Input: part model. Units: mm. Frame: model coordinates. Face numbers are marked on the shaded views. A direction names the side the tool comes from. Round coordinates to 2 decimals unless told otherwise and drop trailing zeros. Order: outer loops, then holes, each group sorted by start corner. A loop starts at its lowest first (then second) coordinate and runs counter-clockwise, first axis right, second up. Notation, with made-up numbers: (-28, 85.25) -> (16, 85.25) arc R22 ccw to (16, 115.25) -> close; hole circle Ø8 at (73, -8.5). An arc over 180 degrees is marked (long way). Use a Markdown table: item, result.
from build123d import *

# Parameters (mm, degrees)
BASE_PLATE_DEPTH           = 580
MOUNTING_HOLES_SKETCH_R    = 5.7
MOUNTING_HOLES_8X_11_DEPTH = 580
HOLE_CHAMFERS_6MM_SIZE     = 9.8


with BuildPart() as part:
    # Plate Profile Sketch → Base Plate (new body)
    with BuildSketch(Plane(origin=(0, 0, 0), x_dir=(0, 0, -1), z_dir=(1, 0, 0))):
        Polygon((-68.5, 0), (68.5, 0), (68.5, 10), (124, 10), (124, 40), (-124, 40), (-124, 10), (-68.5, 10), align=None)
    extrude(amount=BASE_PLATE_DEPTH)

    # Mounting Holes Sketch → Mounting Holes 8xØ11 (cut)
    with BuildSketch(Plane(origin=(0, 40, 0), x_dir=(1, 0, 0), z_dir=(0, 1, 0))):
        with Locations(Location((25, -91.5, 0), (0, 0, 270))):
            Circle(MOUNTING_HOLES_SKETCH_R)
        with Locations(Location((157.5, -91.5, 0), (0, 0, 270))):
            Circle(MOUNTING_HOLES_SKETCH_R)
        with Locations(Location((422.5, -91.5, 0), (0, 0, 270))):
            Circle(MOUNTING_HOLES_SKETCH_R)
        with Locations(Location((555, -91.5, 0), (0, 0, 270))):
            Circle(MOUNTING_HOLES_SKETCH_R)
        with Locations(Location((290, -91.5, 0), (0, 0, 270))):
            Circle(MOUNTING_HOLES_SKETCH_R)
        with Locations(Location((555, 91.5, 0), (0, 0, 270))):
            Circle(MOUNTING_HOLES_SKETCH_R)
        with Locations(Location((422.5, 91.5, 0), (0, 0, 270))):
            Circle(MOUNTING_HOLES_SKETCH_R)
        with Locations(Location((290, 91.5, 0), (0, 0, 270))):
            Circle(MOUNTING_HOLES_SKETCH_R)
        with Locations(Location((157.5, 91.5, 0), (0, 0, 270))):
            Circle(MOUNTING_HOLES_SKETCH_R)
        with Locations(Location((25, 91.5, 0), (0, 0, 270))):
            Circle(MOUNTING_HOLES_SKETCH_R)
    extrude(amount=-MOUNTING_HOLES_8X_11_DEPTH, mode=Mode.SUBTRACT)

    # Hole Chamfers 6mm
    hole_chamfers_6mm_edges = [part.edges().sort_by_distance(p)[0] for p in [
        (25, 40, -97.2),
        (157.5, 40, -97.2),
        (290, 40, -97.2),
        (422.5, 40, -97.2),
        (555, 40, -97.2),
        (157.5, 40, 85.8),
        (422.5, 40, 85.8),
        (555, 40, 85.8),
        (290, 40, 85.8),
        (25, 40, 85.8),
    ]]
    chamfer(hole_chamfers_6mm_edges, length=HOLE_CHAMFERS_6MM_SIZE)


solid = part.part
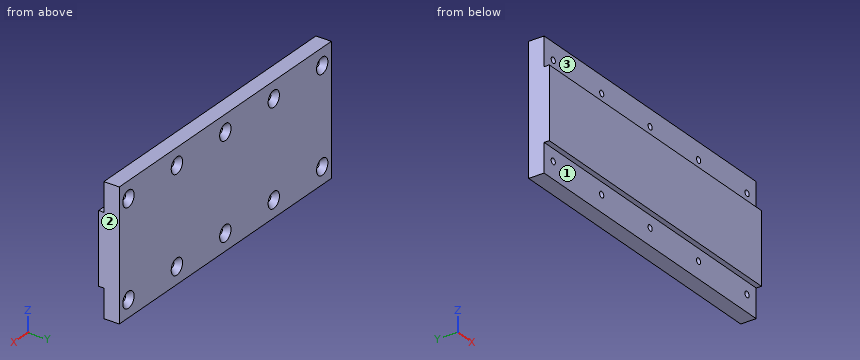
1) Cut plane B-B on z = 91.5. State how many separate pieces and enclosed holes the cut face has, and give its area (3 significant figures).
Answer key:
| item | result |
|---|---|
| separate pieces | 6 |
| enclosed holes | 0 |
| area | 15,200 mm^2 |
2) Cut plane A-A on x = 422.5. Return loops of the section in (y, z).
Answer key:
| item | result |
|---|---|
| outline | (0, -68.5) -> (10, -68.5) -> (10, -85.8) -> (30.2, -85.8) -> (40, -76) -> (40, 76) -> (30.2, 85.8) -> (10, 85.8) -> (10, 68.5) -> (0, 68.5) -> close; (10, -124) -> (40, -124) -> (40, -107) -> (30.2, -97.2) -> (10, -97.2) -> close; (10, 97.2) -> (30.2, 97.2) -> (40, 107) -> (40, 124) -> (10, 124) -> close |
3) Cut plane C-C on x = 88. Return loops of the section in (y, z).
Answer key:
| item | result |
|---|---|
| outline | (0, -68.5) -> (10, -68.5) -> (10, -124) -> (40, -124) -> (40, 124) -> (10, 124) -> (10, 68.5) -> (0, 68.5) -> close |
4) Ray query, probe 1 along X at (y, z) = (18, -91.5); probe 2 along Z at (x, y) = (422.5, 20.5); probe 3 along Z at (x, y) = (156.5, 7). Return the intervals inside material, ascending.
Answer key:
| item | result |
|---|---|
| probe 1 | x = 0 to 19.3, 30.7 to 151.8, 163.2 to 284.3, 295.7 to 416.8, 428.2 to 549.3, 560.7 to 580 |
| probe 2 | z = -124 to -97.2, -85.8 to 85.8, 97.2 to 124 |
| probe 3 | z = -68.5 to 68.5 |
5) Contact query for flat-ended pins moving along their axis: P1, Ø11, axis at x = 254.5, y = 3, coming from the +Z side; P2, Ø18, axis at x = 422.5, z = -91.5, coming from the +Y side; P3, Ø18, axis at x = 422.5, z = 91.5, coming from the -Y side. Output: stop coordinate, or through.
Answer key:
| item | result |
|---|---|
| P1 | stops at z = 68.5 |
| P2 | stops at y = 33.5 |
| P3 | stops at y = 10 |
6) Set-up query: the marked faces 1, 2 and 3. Return all of +Z, -Z, +X, -X, +Y, -Y with unobstructed straight access to the full face (end or side cutting, diameter ignored); none if empty.
Answer key:
| item | result |
|---|---|
| face 1 | -Z, +X, -X, -Y |
| face 2 | +Z, -Z, +X, +Y, -Y |
| face 3 | +Z, +X, -X, -Y |
